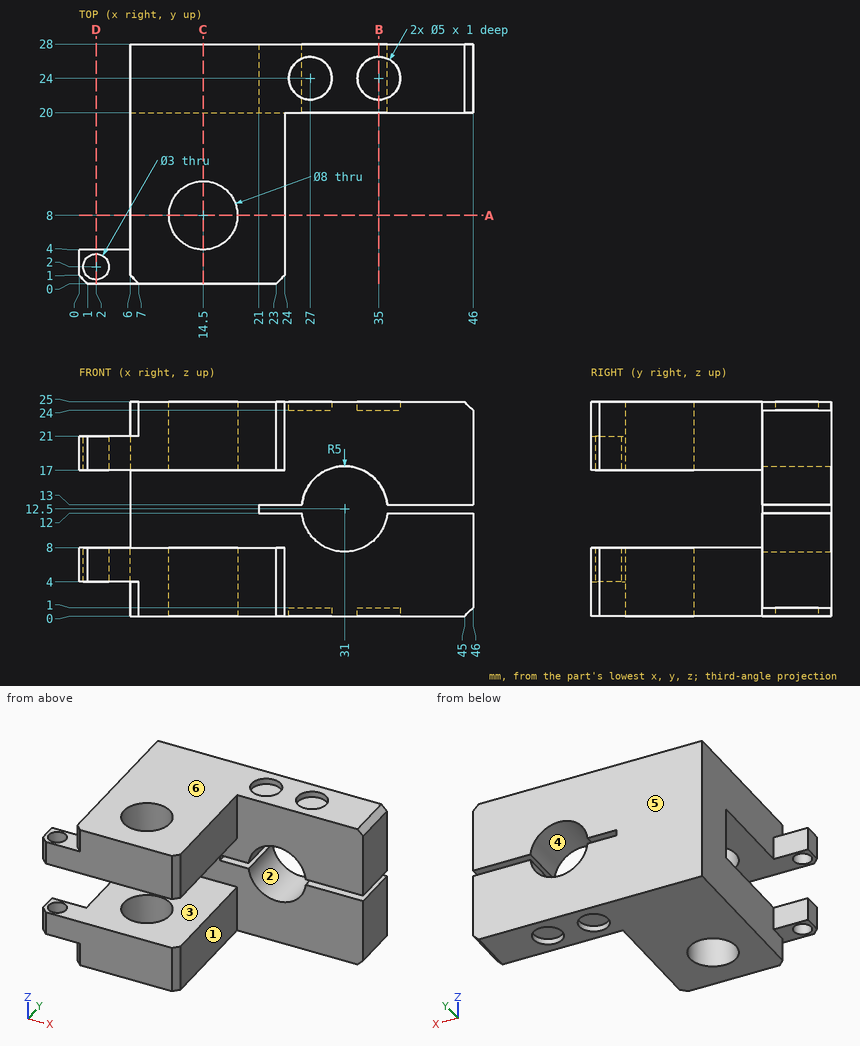
Design review of the part shown in the three views and the two pictorial views. Dimensions are in mm from the part's minimum x, y and z. A direction names the side the tool comes from. Round coordinates to 2 decimals unless told otherwise and drop trailing zeros. Loops run counter-clockwise (first coordinate to the right, second up) from the corner with the lowest first, then second, coordinate; pieces in that order, holes last.
1) Consider section C-C on x = 14.5. State the section outline as (y, z) points.
Values follow:
outline: (0, 0) - (4, 0) - (4, 8) - (0, 8) - close; (0, 17) - (4, 17) - (4, 25) - (0, 25) - close; (12, 0) - (28, 0) - (28, 25) - (12, 25) - (12, 17) - (20, 17) - (20, 8) - (12, 8) - close
2) Consider section B-B on x = 35. State the section outline as (y, z) points, then the cut area to 3 significant figures.
Values follow:
outline: (20, 0) - (21.5, 0) - (21.5, 1) - (26.5, 1) - (26.5, 0) - (28, 0) - (28, 9.5) - (20, 9.5) - close; (20, 15.5) - (28, 15.5) - (28, 25) - (26.5, 25) - (26.5, 24) - (21.5, 24) - (21.5, 25) - (20, 25) - close
area: 142 mm2
3) Consider section A-A on y = 8. State the section outline as (x, z) points, then the cut area to 3 significant figures.
Values follow:
outline: (6, 0) - (10.5, 0) - (10.5, 8) - (6, 8) - close; (6, 17) - (10.5, 17) - (10.5, 25) - (6, 25) - close; (18.5, 0) - (24, 0) - (24, 8) - (18.5, 8) - close; (18.5, 17) - (24, 17) - (24, 25) - (18.5, 25) - close
area: 160 mm2
4) The part is to be moulded in two halves that separate along Z. For the marked faces 4, 5 and 6, say which applies: pulls with the +Z half, pulls with the -Z half, needs draft (parallel to the pull), parting line crosses it, or undercut.
Values follow:
face 4: undercut
face 5: needs draft
face 6: pulls with the +Z half
5) Wall thickness on line 1 along Z through (x, y) = (21, 16.5); line 2 along X through (y, z) = (24, 24.65); line 3 along Z through (x, y) = (44.5, 24.5): over which ranges is each line inside the solid? List them lowest first.
Values follow:
line 1: z = 0 to 8, 17 to 25
line 2: x = 6 to 24.5, 29.5 to 32.5, 37.5 to 45.35
line 3: z = 0 to 12, 13 to 25
6) Clearance check with flat-ended pins moving along their axes: P1, Ø12, axis at y = 21, z = 18, coming from the -X side; P2, Ø6.5, axis at y = 6, z = 6, coming from the +X side; P3, Ø4.5, axis at x = 27, y = 24, coming from the +Z side; P4, Ø5, axis at x = 20.5, z = 16, coming from the -Y side. State where each tip first meets the part, or that it passes through.
Values follow:
P1: stops at x = 6
P2: stops at x = 24
P3: stops at z = 24
P4: stops at y = 0
7) Consider section D-D on x = 2. State the section outline as (y, z) points, then the cut area to 3 significant figures.
Values follow:
outline: (0, 4) - (0.5, 4) - (0.5, 8) - (0, 8) - close; (0, 17) - (0.5, 17) - (0.5, 21) - (0, 21) - close; (3.5, 4) - (4, 4) - (4, 8) - (3.5, 8) - close; (3.5, 17) - (4, 17) - (4, 21) - (3.5, 21) - close
area: 8.00 mm2
8) Tool access review of the marked faces 1, 2 and 3: name each direction out of +Z, -Z, +X, -X, +Y, -Y from which nothing blocks a thin tool from reaching the whole face with its end or side.
Values follow:
face 1: +Z, -Z, +X, -Y
face 2: +Y, -Y
face 3: +X, -X, -Y
